Geometry check sheet. Reference: drawing and pictorial views, mm from the part's lowest x, y, z. A direction names the side the tool comes from. Coordinates: 2 decimals unless noted, no trailing zeros. Write each loop counter-clockwise with the first axis right and the second up, starting at its lowest first coordinate (ties: lowest second). Pieces come first, ordered by that corner, then holes. Notation, with made-up numbers: (15.25, 60.25) -> (28.25, 60.25) arc R29 ccw to (28.25, 81.25) -> close; hole circle Ø2 at (2, 47.5). An arc over 180 degrees is marked (long way). Answer in a Markdown table with one row per item.
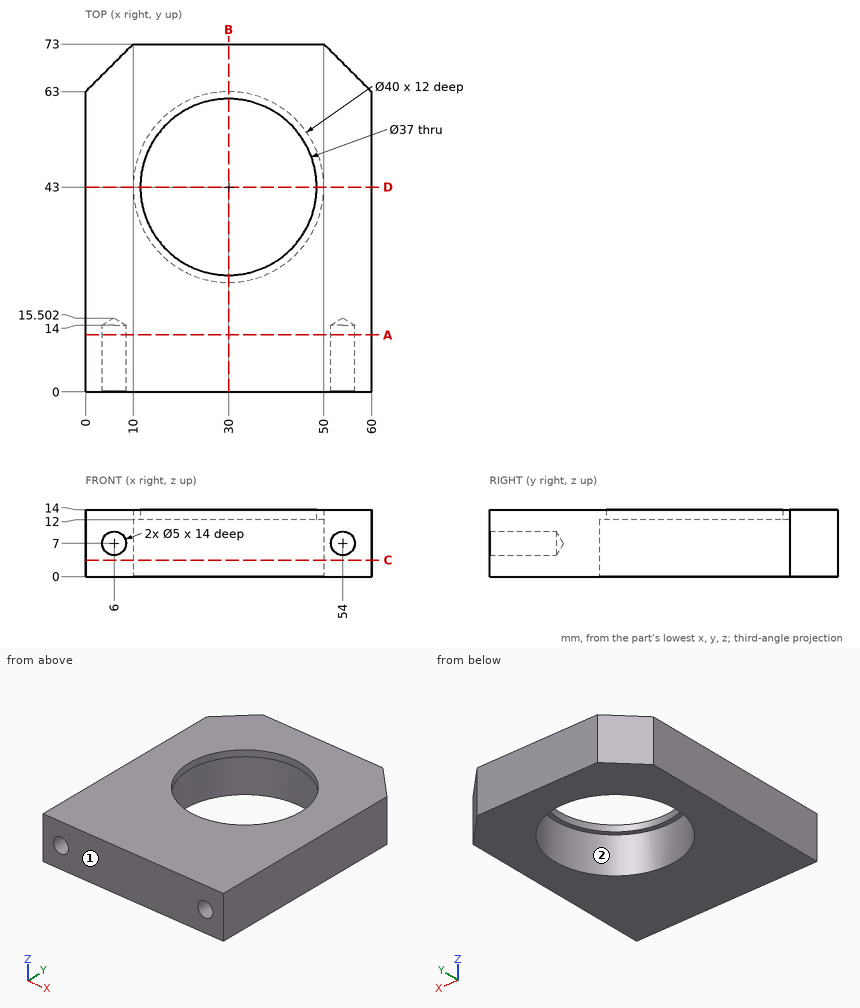
1. Thickness scan on line 1 (X direction, y = 5.5, z = 7); line 2 (Y direction, x = 30, z = 8.75); line 3 (Z direction, x = 6, y = 6.75). Record the ranges inside material, lowest first. Write a range as from..to.
Geometry says:
| item | result |
|---|---|
| line 1 | 0..3.5, 8.5..51.5, 56.5..60 |
| line 2 | 0..23, 63..73 |
| line 3 | 0..4.5, 9.5..14 |
2. Section check D-D, the plane y = 43. Record the boundary of the cut face in (x, z), plus the area to 3 significant figures.
Geometry says:
| item | result |
|---|---|
| outline | (0, 0) -> (10, 0) -> (10, 12) -> (11.5, 12) -> (11.5, 14) -> (0, 14) -> close; (48.5, 12) -> (50, 12) -> (50, 0) -> (60, 0) -> (60, 14) -> (48.5, 14) -> close |
| area | 286 mm^2 |
3. Section check B-B, the plane x = 30. Record the boundary of the cut face in (y, z), plus the area to 3 significant figures.
Geometry says:
| item | result |
|---|---|
| outline | (0, 0) -> (23, 0) -> (23, 12) -> (24.5, 12) -> (24.5, 14) -> (0, 14) -> close; (61.5, 12) -> (63, 12) -> (63, 0) -> (73, 0) -> (73, 14) -> (61.5, 14) -> close |
| area | 468 mm^2 |
4. Section check C-C, the plane z = 3.5. Record the boundary of the cut face in (x, y).
Geometry says:
| item | result |
|---|---|
| outline | (0, 0) -> (60, 0) -> (60, 63) -> (50, 73) -> (10, 73) -> (0, 63) -> close; hole circle Ø40 at (30, 43) |
5. Section check A-A, the plane y = 12. Record the boundary of the cut face in (x, z).
Geometry says:
| item | result |
|---|---|
| outline | (0, 0) -> (60, 0) -> (60, 14) -> (0, 14) -> close; hole circle Ø5 at (6, 7); hole circle Ø5 at (54, 7) |
6. Tool access check on the marked faces 1 and 2. Record the directions out of +Z, -Z, +X, -X, +Y, -Y that give a thin tool (end or side, any length) a straight path to the whole face; none if there is none.
Geometry says:
| item | result |
|---|---|
| face 1 | +Z, -Z, +X, -X, -Y |
| face 2 | -Z |
7. Depth check by flat-ended pin: P1, Ø4.5, axis at x = 6, z = 7, coming from the +Y side. Enter the tip coordinate at first touch or a pass-through.
Geometry says:
| item | result |
|---|---|
| P1 | y = 71.25 |
